```python
from build123d import *

# Parameters (mm, degrees)
SKETCH_1_R      = 30
EXTRUDE_1_DEPTH = 70
SKETCH_2_R      = 37.5
EXTRUDE_2_DEPTH = 20
CHAMFER_2_SIZE  = 2
SKETCH_3_W      = 1
SKETCH_3_H      = 2


with BuildPart() as part:
    # 草图1 → 凸台-拉伸1 (new body)
    with BuildSketch(Plane.XY):
        Circle(SKETCH_1_R)
    extrude(amount=EXTRUDE_1_DEPTH)

    # 草图2 → 凸台-拉伸2 (add)
    with BuildSketch(Plane.XY.offset(70)):
        Circle(SKETCH_2_R)
    extrude(amount=EXTRUDE_2_DEPTH)

    # 倒角2
    chamfer_2_edges = [part.edges().sort_by_distance(p)[0] for p in [
        (-30, 0, 0),
    ]]
    chamfer(chamfer_2_edges, length=CHAMFER_2_SIZE)

    # 草图3 → 切除-旋转1 (revolve, cut)
    with BuildSketch(Plane(origin=(0, 0, 0), x_dir=(1, 0, 0), z_dir=(0, 1, 0))):
        with Locations((29.5, -69)):
            Rectangle(SKETCH_3_W, SKETCH_3_H)
    revolve(axis=Axis((0, 0, 70), (0, 0, -1)), mode=Mode.SUBTRACT)


solid = part.part
```
Here's how the part is built. I have some questions about the finished solid (model axes, mm). A direction names the side the tool comes from. Give positions to 0.01 mm unless a question says otherwise; leave off trailing zeros. Order: outer loops, then holes, each group sorted by start corner. A loop starts at its lowest first (then second) coordinate and runs counter-clockwise, first axis right, second up. Notation, with made-up numbers: M 28,12 L 49,12 A5 ccw 49,18 Z; hole C 12,18.5 d9. An arc over 180 degrees is marked long. Use a Markdown table: item, result. Add a question column.
1. Suppose I cut it at A-A (x = 0). List the corners of the cut face in (y, z) for me.
2. For pin 1 Ø4 at (x, z) = (-4.5, 72) entering from +Y; pin 2 Ø10 at (x, z) = (24.5, 71) entering from -Y; pin 3 Ø5 at (y, z) = (24, 73) entering from -X, each with a flat end and sliding along its axis, tell me the tip position at first contact or that it passes through.
3. I need wall thicknesses on probe 1 along Z at (x, y) = (20, -24); probe 2 along X at (y, z) = (0.5, 56.5); probe 3 along X at (y, z) = (-1, 79.5). Which ranges of each line are inside material? Lowest first, please. Write a range as from..to.
4. Suppose I cut it at C-C (z = 38). List the corners of the cut face in (x, y) for me, and give its area (3 significant figures).
5. If we mould it in two halves opening along Z, with no side actions, what happens to faces 1 (the cylindrical face through (13.38, 25.73, 68.99)), 2 (the flat face through (16, -25, 68)), 3 (the flat face through (-1, 1, 90)), 4 (the cylindrical face through (-4.88, 37.18, 79.86))? For each: +Z half, -Z half, draft (parallel to the pull), parting line (faces both ways), or undercut.
6. Suppose I cut it at D-D (y = 32). List the corners of the cut face in (x, z) for me, and give its area (3 significant figures).
7. On a 3-axis mill with a long thin cutter (end or side, diameter ignored), from which of +Z, -Z, +X, -X, +Y, -Y can I reach the whole of each face in a straight line? I mean faces 5 (the cylindrical face through (-29.97, 1.32, 34.54)), 6 (the flat face through (0, 0, 0)). Say none if no direction works.
Results list:
| question | item | result |
|---|---|---|
| 1 | outline | M -37.5,70 L -29,70 L -29,68 L -30,68 L -30,2 L -28,0 L 28,0 L 30,2 L 30,68 L 29,68 L 29,70 L 37.5,70 L 37.5,90 L -37.5,90 Z |
| 2 | pin 1 | stops at y = 37.42 |
| 2 | pin 2 | stops at y = -32.03 |
| 2 | pin 3 | stops at x = -30.72 |
| 3 | probe 1 | z = 70..90 |
| 3 | probe 2 | x = -30..30 |
| 3 | probe 3 | x = -37.49..37.49 |
| 4 | outline | C 0,0 d60 |
| 4 | area | 2,830 mm² |
| 5 | face 1 | undercut |
| 5 | face 2 | undercut |
| 5 | face 3 | +Z half |
| 5 | face 4 | draft |
| 6 | outline | M -19.55,70 L 19.55,70 L 19.55,90 L -19.55,90 Z |
| 6 | area | 782 mm² |
| 7 | face 5 | -Z |
| 7 | face 6 | -Z, +X, -X, +Y, -Y |
